```python
from build123d import *

# Parameters (mm, degrees)
BOSS_EXTRUDE1_DEPTH = 15
CUT_EXTRUDE1_START  = -10
CUT_EXTRUDE1_DEPTH  = 10
BOSS_EXTRUDE3_START = -5
BOSS_EXTRUDE3_DEPTH = 5
SKETCH5_R           = 1
CUT_EXTRUDE2_DEPTH  = 15
CUT_EXTRUDE4_START  = -15
CUT_EXTRUDE4_DEPTH  = 15
CUT_EXTRUDE5_START  = -15
CUT_EXTRUDE5_DEPTH  = 15


with BuildPart() as part:
    # Sketch1 → Boss-Extrude1 (new body)
    with BuildSketch(Plane.XY):
        with BuildLine():
            Line((6.964115375, 114.788941528), (9.188776982, 134.686919846))
            ThreePointArc((9.188776982, 134.686919846), (21.482610172, 133.279771384), (33.595955959, 130.752865143))
            Line((33.595955959, 130.752865143), (26.130187968, 101.696672889))
            ThreePointArc((26.130187968, 101.696672889), (21.669371251, 102.739662982), (17.167305653, 103.587082286))
            Line((17.167305653, 103.587082286), (18.802287144, 113.452518695))
            ThreePointArc((18.802287144, 113.452518695), (12.90051864, 114.274129263), (6.964115375, 114.788941528))
        make_face()
    extrude(amount=BOSS_EXTRUDE1_DEPTH)

    # Sketch3 → Cut-Extrude1 (cut)
    with BuildSketch(Plane.XY.offset(15).offset(CUT_EXTRUDE1_START)):
        with BuildLine():
            ThreePointArc((18.802287144, 113.452518695), (23.733120893, 112.52439279), (28.618777298, 111.382070307))
            Line((28.618777298, 111.382070307), (31.107147965, 121.066616705))
            ThreePointArc((31.107147965, 121.066616705), (19.677605268, 123.440561348), (8.076446178, 124.737930687))
            Line((8.076446178, 124.737930687), (6.964115375, 114.788941528))
            ThreePointArc((6.964115375, 114.788941528), (12.90051864, 114.274129263), (18.802287144, 113.452518695))
        make_face()
    extrude(amount=CUT_EXTRUDE1_DEPTH, mode=Mode.SUBTRACT)

    # Sketch4 → Boss-Extrude3 (add)
    with BuildSketch(Plane.XY.offset(15).offset(BOSS_EXTRUDE3_START)):
        with BuildLine():
            ThreePointArc((28.618777298, 111.382070307), (17.872807715, 113.602652893), (6.964115375, 114.788941528))
            Line((6.964115375, 114.788941528), (8.076446178, 124.737930687))
            ThreePointArc((8.076446178, 124.737930687), (19.677605268, 123.440561348), (31.107147965, 121.066616705))
            Line((31.107147965, 121.066616705), (28.618777298, 111.382070307))
        make_face()
    extrude(amount=BOSS_EXTRUDE3_DEPTH)

    # Sketch5 → Cut-Extrude2 (cut)
    with BuildSketch(Plane.XY.offset(15)):
        with Locations((25.988912996, 117.220204748)):
            Circle(SKETCH5_R)
    extrude(amount=-CUT_EXTRUDE2_DEPTH, mode=Mode.SUBTRACT)

    # Sketch7 → Cut-Extrude4 (cut)
    with BuildSketch(Plane.XY.offset(15).offset(CUT_EXTRUDE4_START)):
        with BuildLine():
            Line((0, 115), (0, 135))
            ThreePointArc((0, 135), (8.829422446, 134.710954637), (17.62103595, 133.845056285))
            Line((17.62103595, 133.845056285), (15.010512105, 114.016159058))
            ThreePointArc((15.010512105, 114.016159058), (7.521359861, 114.753776172), (0, 115))
        make_face()
    extrude(amount=CUT_EXTRUDE4_DEPTH, mode=Mode.SUBTRACT)

    # Sketch8 → Cut-Extrude5 (cut)
    with BuildSketch(Plane.XY.offset(15).offset(CUT_EXTRUDE5_START)):
        with BuildLine():
            Line((15.010512105, 114.016159058), (15.663143066, 118.973383365))
            ThreePointArc((15.663143066, 118.973383365), (17.643911325, 118.695797706), (19.619777889, 118.385236899))
            Line((19.619777889, 118.385236899), (18.802287144, 113.452518695))
            ThreePointArc((18.802287144, 113.452518695), (16.908748354, 113.750139469), (15.010512105, 114.016159058))
        make_face()
    extrude(amount=CUT_EXTRUDE5_DEPTH, mode=Mode.SUBTRACT)


solid = part.part
```
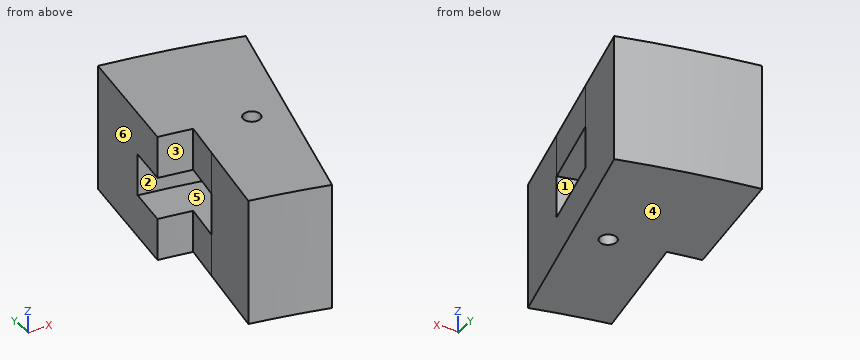
Check sheet for the modelled part. Datum: model origin and axes. Units: mm. Face numbers are marked on the shaded views. A direction names the side the tool comes from. Round coordinates to 2 decimals unless told otherwise and drop trailing zeros. Loops run counter-clockwise (first coordinate to the right, second up) from the corner with the lowest first, then second, coordinate; pieces in that order, holes last. Notation, with made-up numbers: (-32.5, -29.75) - (-12.5, -29.75) arc R34 cw to (-12.5, 0.25) - close; hole circle Ø8 at (-22.75, -19). An arc over 180 degrees is marked (long way). Answer as a JSON object with one key per item and string values. Group by question number.
Q1. Scan lines: line 1 along Z through (x, y) = (27.5, 113); line 2 along Y through (x, z) = (24.5, 9.25); line 3 along Y through (x, z) = (26, 4.75). Record each from-to range of solid material in increasing order. Write a range as [from, to].
Q2. Mould release check, pull along Y, two halves, no side actions. Record for the marked faces 4, 5 and 6: released by +Y, released by -Y, zero draft, split by the parting line, or undercut.
Q3. Sectioned sample at A-A, the plane z = 9.25. Enter the section's corners in (x, y).
Q4. Sectioned sample at B-B, the plane x = 23. Enter the section's corners in (y, z), plus the area to 3 significant figures.
Q5. Gauge pin test, flat ends, axial feed: P1, Ø8, axis at y = 110, z = 3.5, coming from the +X side; P2, Ø1.6, axis at x = 25.99, y = 117.22, coming from the -Z side; P3, Ø8, axis at y = 114, z = 9, coming from the -X side; P4, Ø1.5, axis at y = 115, z = 10, coming from the +X side. Record the tip position at first contact, or that the pin passes through.
Q6. Set-up check for the marked faces 1, 2 and 3: record each of +Z, -Z, +X, -X, +Y, -Y from which the full face is reachable in a straight line by a thin tool's end or side.
Q7. Sectioned sample at D-D, the plane y = 110.5. Enter the section's corners in (x, z), plus the area to 3 significant figures.
Q8. Sectioned sample at C-C, the plane z = 13.5. Enter the section's corners in (x, y), plus the area to 3 significant figures.
Solution:
{
 "1": {"line 1": "z = [0, 5], [10, 15]", "line 2": "y = [102.1, 112.36], [122.57, 132.76]", "line 3": "y = [101.73, 116.22], [118.22, 132.47]"},
 "2": {"face 4": "zero draft", "face 5": "undercut", "face 6": "released by +Y"},
 "3": {"outline": "(16.32, 123.93) arc R125 cw to (31.11, 121.07) - (33.6, 130.75) arc R135 ccw to (17.62, 133.85) - close; (17.17, 103.59) arc R105 cw to (26.13, 101.7) - (28.62, 111.38) arc R115 ccw to (18.8, 113.45) - close"},
 "4": {"outline": "(102.45, 0) - (133.03, 0) - (133.03, 15) - (102.45, 15) - close; hole (112.68, 5) - (122.86, 5) - (122.86, 10) - (112.68, 10) - close", "area": "408 mm²"},
 "5": {"P1": "stops at x = 29.29", "P2": "passes through", "P3": "stops at x = 18.23", "P4": "stops at x = 29.74"},
 "6": {"face 1": "+X", "face 2": "-X", "face 3": "+Z, -Z, -X"},
 "7": {"outline": "(18.31, 0) - (28.39, 0) - (28.39, 15) - (18.31, 15) - close", "area": "151 mm²"},
 "8": {"outline": "(15.66, 118.97) arc R120 cw to (19.62, 118.39) - (17.17, 103.59) arc R105 cw to (26.13, 101.7) - (33.6, 130.75) arc R135 ccw to (17.62, 133.85) - close; hole circle Ø2 at (25.99, 117.22)", "area": "375 mm²"}
}
